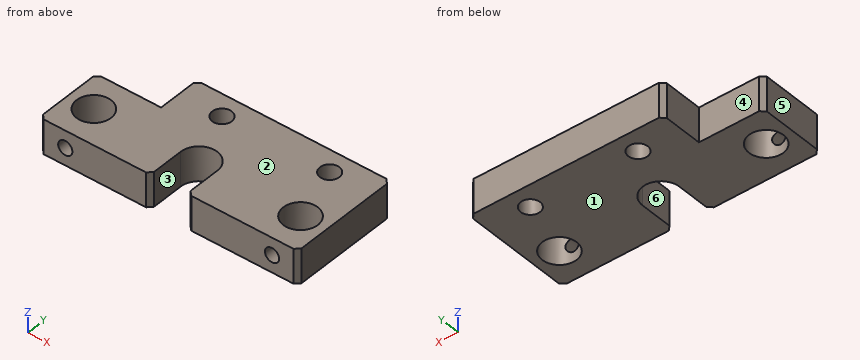
from build123d import *

# Parameters (mm, degrees)
SKETCH1_W              = 60
SKETCH1_H              = 26
SKETCH1_R              = 4
BOSS_EXTRUDE1_DEPTH    = 8
CUT_EXTRUDE1_DEPTH     = 41.496913463
M4_TAPPED_HOLE1_REACH  = 42.497
M4_TAPPED_HOLE1_BORE_R = 1.65
SKETCH8_W              = 15
SKETCH8_H              = 10
CUT_EXTRUDE2_DEPTH     = 41.496913482
SKETCH9_R              = 2.25
CUT_EXTRUDE3_DEPTH     = 41.496913482
CHAMFER1_SIZE          = 1


with BuildPart() as part:
    # Sketch1 → Boss-Extrude1 (new body)
    with BuildSketch(Plane.XY):
        with Locations((0, 13)):
            Rectangle(SKETCH1_W, SKETCH1_H)
        with Locations((-24, 8)):
            Circle(SKETCH1_R, mode=Mode.SUBTRACT)
        with Locations(Location((24, 8, 0), (0, 0, 180))):
            Circle(SKETCH1_R, mode=Mode.SUBTRACT)
    extrude(amount=BOSS_EXTRUDE1_DEPTH)

    # Sketch2 → Cut-Extrude1 (cut, through all)
    with BuildSketch(Plane.XY.offset(8)):
        with BuildLine():
            Line((-4.25, 0), (-4.25, 8.5))
            ThreePointArc((-4.25, 8.5), (0, 12.75), (4.25, 8.5))
            Line((4.25, 8.5), (4.25, 0))
            ThreePointArc((4.25, 0), (0, -4.25), (-4.25, 0))
        make_face()
    extrude(amount=-CUT_EXTRUDE1_DEPTH, mode=Mode.SUBTRACT)

    # M4 Tapped Hole1 bore → M4 Tapped Hole1 (cut, up to next)
    with BuildSketch(Plane.XZ, mode=Mode.PRIVATE) as m4_tapped_hole1_sk1:
        with Locations((-24, 4)):
            Circle(M4_TAPPED_HOLE1_BORE_R)
    m4_tapped_hole1_tool1 = extrude(m4_tapped_hole1_sk1.sketch, amount=-M4_TAPPED_HOLE1_REACH, mode=Mode.PRIVATE) & part.part
    # M4 Tapped Hole1 bore → M4 Tapped Hole1 (cut, up to next)
    with BuildSketch(Plane.XZ, mode=Mode.PRIVATE) as m4_tapped_hole1_sk2:
        with Locations((24, 4)):
            Circle(M4_TAPPED_HOLE1_BORE_R)
    m4_tapped_hole1_tool2 = extrude(m4_tapped_hole1_sk2.sketch, amount=-M4_TAPPED_HOLE1_REACH, mode=Mode.PRIVATE) & part.part
    add(m4_tapped_hole1_tool1.solids().sort_by_distance((-24, 0, 4))[0], mode=Mode.SUBTRACT)
    add(m4_tapped_hole1_tool2.solids().sort_by_distance((24, 0, 4))[0], mode=Mode.SUBTRACT)

    # Sketch8 → Cut-Extrude2 (cut, through all)
    with BuildSketch(Plane(origin=(0, 0, 0), x_dir=(-1, 0, 0), z_dir=(0, 0, -1))):
        with Locations((22.5, 21)):
            Rectangle(SKETCH8_W, SKETCH8_H)
    extrude(amount=-CUT_EXTRUDE2_DEPTH, mode=Mode.SUBTRACT)

    # Sketch9 → Cut-Extrude3 (cut, through all)
    with BuildSketch(Plane(origin=(0, 0, 0), x_dir=(-1, 0, 0), z_dir=(0, 0, -1))):
        with Locations((-20, 21)):
            Circle(SKETCH9_R)
        with Locations((5, 21)):
            Circle(SKETCH9_R)
    extrude(amount=-CUT_EXTRUDE3_DEPTH, mode=Mode.SUBTRACT)

    # Chamfer1
    chamfer1_edges = [part.edges().sort_by_distance(p)[0] for p in [
        (4.25, 0, 4),
        (-4.25, 0, 4),
        (-15, 26, 4),
        (-30, 16, 4),
        (30, 0, 4),
        (-30, 0, 4),
        (30, 26, 4),
    ]]
    chamfer(chamfer1_edges, length=CHAMFER1_SIZE)


solid = part.part
CAD build for the part. Positions are in the model's coordinates, mm. Face numbers are marked on the shaded views. A direction names the side the tool comes from. Round coordinates to 2 decimals unless told otherwise and drop trailing zeros. Write each loop counter-clockwise with the first axis right and the second up, starting at its lowest first coordinate (ties: lowest second). Pieces come first, ordered by that corner, then holes. Notation, with made-up numbers: M 70.5,25 L 74.5,25 A19 cw 74.5,36 Z; hole C -28.5,71 d9. An arc over 180 degrees is marked long. Use a Markdown table: item, result. Add a question column.
1. 3-axis set-ups, long thin cutter, end or side, ignore diameter. For the marked faces 4, 5 and 6: which of +Z, -Z, +X, -X, +Y, -Y reach the whole face in a straight line?
2. Slice it at B-B on y = 21. Give the cut face in (x, z), then the cut area to 3 significant figures.
3. Slice it at C-C on x = 24. Give the cut face in (y, z), then the cut area to 3 significant figures.
4. Pull direction Z, two halves, no side cores. Call the marked faces 1, 2 and 3: released by +Z, released by -Z, zero draft, split by the parting line, or undercut.
5. Slice it at A-A on z = 7. Give the cut face in (x, y), then the cut area to 3 significant figures.
6. Slice it at D-D on z = 4. Give the cut face in (x, y).
7. Drill centre lines: probe 1 along X at (y, z) = (2.6, 4); probe 2 along X at (y, z) = (8.25, 7.75); probe 3 along Z at (x, y) = (24, 3.3). Where is each one in solid material? Low to high.
8. Flat gauge pins, fed straight in: P1, Ø2, axis at x = 24, z = 4, coming from the -Y side; P2, Ø2.5, axis at x = 20, y = 21, coming from the -Z side; P3, Ø1.5, axis at x = -5, y = 16.5, coming from the -Z side; P4, Ø2, axis at x = -19.5, z = 2.5, coming from the +Y side. Where does each tip first touch, or does it go through?
Reply:
| question | item | result |
|---|---|---|
| 1 | face 4 | +Z, -Z, -X, +Y |
| 1 | face 5 | +Z, -Z, -X, +Y, -Y |
| 1 | face 6 | +Z, -Z, -Y |
| 2 | outline | M -15,0 L -7.25,0 L -7.25,8 L -15,8 Z; M -2.75,0 L 17.75,0 L 17.75,8 L -2.75,8 Z; M 22.25,0 L 30,0 L 30,8 L 22.25,8 Z |
| 2 | area | 288 mm^2 |
| 3 | outline | M 0,0 L 4,0 L 4,2.35 L 0,2.35 Z; M 0,5.65 L 4,5.65 L 4,8 L 0,8 Z; M 12,0 L 26,0 L 26,8 L 12,8 Z |
| 3 | area | 131 mm^2 |
| 4 | face 1 | released by -Z |
| 4 | face 2 | released by +Z |
| 4 | face 3 | zero draft |
| 5 | outline | M -30,1 L -29,0 L -5.25,0 L -4.25,1 L -4.25,8.5 A4.25 cw 4.25,8.5 L 4.25,1 L 5.25,0 L 29,0 L 30,1 L 30,25 L 29,26 L -14,26 L -15,25 L -15,16 L -29,16 L -30,15 Z; hole C -24,8 d8; hole C -5,21 d4.5; hole C 20,21 d4.5; hole C 24,8 d8 |
| 5 | area | 1,170 mm^2 |
| 6 | outline | M -30,1 L -29,0 L -25.65,0 L -25.65,4.36 A4 cw long -22.35,4.36 L -22.35,0 L -5.25,0 L -4.25,1 L -4.25,8.5 A4.25 cw 4.25,8.5 L 4.25,1 L 5.25,0 L 22.35,0 L 22.35,4.36 A4 cw long 25.65,4.36 L 25.65,0 L 29,0 L 30,1 L 30,25 L 29,26 L -14,26 L -15,25 L -15,16 L -29,16 L -30,15 Z; hole C -5,21 d4.5; hole C 20,21 d4.5 |
| 7 | probe 1 | x = -30 to -25.65, -22.35 to -4.25, 4.25 to 22.35, 25.65 to 30 |
| 7 | probe 2 | x = -30 to -27.99, -20.01 to -4.25, 4.25 to 20.01, 27.99 to 30 |
| 7 | probe 3 | z = 0 to 2.35, 5.65 to 8 |
| 8 | P1 | stops at y = 11.87 |
| 8 | P2 | passes through |
| 8 | P3 | stops at z = 0 |
| 8 | P4 | stops at y = 16 |
